Can you work these out from the model? Positions are in its coordinate system, mm. A direction names the side the tool comes from. Coordinates: 2 decimals unless noted, no trailing zeros. Order: outer loops, then holes, each group sorted by start corner. A loop starts at its lowest first (then second) coordinate and runs counter-clockwise, first axis right, second up. Notation, with made-up numbers: M 23,-25 L 27,-25 A22 ccw 27,-8 Z; hole C -7.5,-10 d10. An arc over 180 degrees is marked long. Answer as a JSON object with one key per item and string values.
from build123d import *

# Parameters (mm, degrees)
BOSS_EXTRUDE1_DEPTH = 130
FILLET1_R           = 3
SKETCH2_R           = 4
CUT_EXTRUDE1_DEPTH  = 130


with BuildPart() as part:
    # Sketch1 → Boss-Extrude1 (new body)
    with BuildSketch(Plane.XY):
        Polygon((0, 0), (40, 0), (40, -40), (36, -40), (36, -4), (0, -4), align=None)
    extrude(amount=BOSS_EXTRUDE1_DEPTH)

    # Fillet1
    fillet1_edges = [part.edges().sort_by_distance(p)[0] for p in [
        (0, -4, 65),
        (36, -4, 65),
        (36, -40, 65),
    ]]
    fillet(fillet1_edges, radius=FILLET1_R)

    # Sketch2 → Cut-Extrude1 (cut)
    with BuildSketch(Plane.XZ.offset(4)):
        with Locations(Location((15, 115, 0), (0, 0, 270))):
            Circle(SKETCH2_R)
        with Locations(Location((15, 15, 0), (0, 0, 270))):
            Circle(SKETCH2_R)
    extrude(amount=-CUT_EXTRUDE1_DEPTH, mode=Mode.SUBTRACT)


solid = part.part
Item 1: I want a section at A-A, the plane x = 15. Write out the boundary of the cut face in (y, z).
Answers follow:
{"outline": "M -4,0 L 0,0 L 0,11 L -4,11 Z; M -4,19 L 0,19 L 0,111 L -4,111 Z; M -4,119 L 0,119 L 0,130 L -4,130 Z"}
Item 2: I want a section at D-D, the plane z = 64. Write out the boundary of the cut face in (x, y), plus the area to 3 significant figures.
Answers follow:
{"outline": "M 0,-1 A3 ccw 3,-4 L 33,-4 A3 cw 36,-7 L 36,-37 A3 ccw 39,-40 L 40,-40 L 40,0 L 0,0 Z", "area": "302 mm^2"}
Item 3: Which directions (+Z, -Z, +X, -X, +Y, -Y) give clear straight access to the entire face, cutting with the end or side of a thin tool? Please do faces 1 (the cylindrical face through (16.201, -2.028, 111.185)), 2 (the flat face through (18, -4, 64)).
Answers follow:
{"face 1": "+Y, -Y", "face 2": "+Z, -Z, -X, -Y"}
Item 4: I want a section at B-B, the plane z = 15. Write out the boundary of the cut face in (x, y), plus the area to 3 significant figures.
Answers follow:
{"outline": "M 0,-1 A3 ccw 3,-4 L 11,-4 L 11,0 L 0,0 Z; M 19,-4 L 33,-4 A3 cw 36,-7 L 36,-37 A3 ccw 39,-40 L 40,-40 L 40,0 L 19,0 Z", "area": "270 mm^2"}
Item 5: I want a section at C-C, the plane y = -2.5. Write out the boundary of the cut face in (x, z).
Answers follow:
{"outline": "M 0.4,0 L 40,0 L 40,130 L 0.4,130 Z; hole C 15,15 d8; hole C 15,115 d8"}
Item 6: I'm going to push flat-ended pins straight in: pin 1 (1 mm diameter, centred on x = 11, z = 50, fed in from -Y); pin 2 (3 mm diameter, centred on x = 21.5, y = -4.5, fed in from +Z); pin 3 (9 mm diameter, centred on y = -23, z = 87, fed in from -X). Where does each tip first touch, or does it pass through?
Answers follow:
{"pin 1": "stops at y = -4", "pin 2": "stops at z = 130", "pin 3": "stops at x = 36"}
Item 7: Please list where these lines run through material, in increasing order: line 1 (X direction, y = -1, z = 115); line 2 (Y direction, x = 26, z = 29); line 3 (X direction, y = -35.5, z = 7).
Answers follow:
{"line 1": "x = 0 to 11, 19 to 40", "line 2": "y = -4 to 0", "line 3": "x = 36 to 40"}
Item 8: If we mould it in two halves opening along Z, with no side actions, what happens to faces 3 (the flat face through (20, 0, 64)), 4 (the flat face through (29, -3.6, 130)), 5 (the cylindrical face through (17.7, -2.03, 17.95))? For each: pulls with the +Z half, pulls with the -Z half, needs draft (parallel to the pull), parting line crosses it, or undercut.
Answers follow:
{"face 3": "needs draft", "face 4": "pulls with the +Z half", "face 5": "undercut"}
